Geometry check sheet. Reference: the model listing, model coordinates, mm. A direction names the side the tool comes from. Give positions to 0.01 mm unless a question says otherwise; leave off trailing zeros. Loops run counter-clockwise (first coordinate to the right, second up) from the corner with the lowest first, then second, coordinate; pieces in that order, holes last. Notation, with made-up numbers: (-4, 28.5) - (4, 28.5) arc R29 ccw to (4, 56.5) - close; hole circle Ø8 at (-20.75, 40.5). An arc over 180 degrees is marked (long way). One line per question, with ' | ' between items. Start each with the question number.
from build123d import *

# Parameters (mm, degrees)
BOSS_EXTRUDE1_DEPTH                          = 3
SKETCH11_R                                   = 1.5
CUT_EXTRUDE1_DEPTH                           = 3
CBORE_FOR_M5_HEXAGON_HEAD_BOLTS_FULL_2_COUNT = 2
CBORE_FOR_M5_HEXAGON_HEAD_BOLTS_FULL_2_PITCH = 40


with BuildPart() as part:
    # Sketch4 → Boss-Extrude1 (new body)
    with BuildSketch(Plane.XY):
        with BuildLine():
            Line((30, 0), (30, -30))
            ThreePointArc((30, -30), (0, -42.426406871), (-30, -30))
            Line((-30, -30), (-30, 0))
            ThreePointArc((-30, 0), (0, 30), (30, 0))
        make_face()
        with BuildLine():
            Line((6.2, 0), (6.2, -15.218791378))
            ThreePointArc((6.2, -15.218791378), (0, -21.418791378), (-6.2, -15.218791378))
            Line((-6.2, -15.218791378), (-6.2, 0))
            ThreePointArc((-6.2, 0), (0, 6.2), (6.2, 0))
        make_face(mode=Mode.SUBTRACT)
    extrude(amount=BOSS_EXTRUDE1_DEPTH)

    # Sketch11 → Cut-Extrude1 (cut)
    with BuildSketch(Plane.XY.offset(3)):
        with Locations((-15.463782922, 0)):
            Circle(SKETCH11_R)
        with Locations((-7.731891461, 13.392028849)):
            Circle(SKETCH11_R)
        with Locations((7.731891461, 13.392028849)):
            Circle(SKETCH11_R)
        with Locations((15.463782922, 0)):
            Circle(SKETCH11_R)
        with Locations((7.731891461, -13.392028849)):
            Circle(SKETCH11_R)
        with Locations((-7.731891461, -13.392028849)):
            Circle(SKETCH11_R)
    extrude(amount=-CUT_EXTRUDE1_DEPTH, mode=Mode.SUBTRACT)

    # Sketch14 → CBORE for M5 Hexagon head bolts-Full thread-grade C1 (revolve, cut)
    with BuildSketch(Plane(origin=(20, -30, 3), x_dir=(0, -1, 0), z_dir=(1, 0, 0))):
        Polygon((0, 0), (0, 3), (2.75, 3), (2.75, 0.5), (5.5, 0.5), (5.5, 0.025), (5.525, 0), align=None)
    cbore_for_m5_hexagon_head_bolts_full_thr = revolve(axis=Axis((20, -30, 9.35), (0, 0, -1)), mode=Mode.SUBTRACT)

    # CBORE for M5 Hexagon head bolts-Full 2: CBORE for M5 Hexagon head bolts-Full thread-grade C1 ×2
    with Locations(*[(-i * CBORE_FOR_M5_HEXAGON_HEAD_BOLTS_FULL_2_PITCH, 0, 0) for i in range(1, CBORE_FOR_M5_HEXAGON_HEAD_BOLTS_FULL_2_COUNT)]):
        add(cbore_for_m5_hexagon_head_bolts_full_thr, mode=Mode.SUBTRACT)


solid = part.part
(1) Section check D-D, the plane x = -20. Record the boundary of the cut face in (y, z) (3 decimals).
(2) Tool access check on faces 4 (the face through (7, -6, 0)), 5 (the face through (0.136, -21.417, 1.479)), 6 (the face through (-23.72, -25.95, 2.74)). Record the directions out of +Z, -Z, +X, -X, +Y, -Y that give a thin tool (end or side, any length) a straight path to the whole face; none if there is none.
(3) Section check B-B, the plane z = 1.95. Count the separate pieces of the cut face and the enclosed holes in it, and give its area (3 significant figures).
(4) Section check A-A, the plane x = 0. Record the boundary of the cut face in (y, z), and give its area (3 significant figures).
(5) Section check C-C, the plane y = 20. Record the boundary of the cut face in (x, z), and give its area (3 significant figures).
(6) Mould release check, pull along X, two halves, no side actions. Record for faces 1 (the face through (7, -6, 3)), 2 (the face through (-0.1, 6.2, 1.5)), 3 (the face through (-0.66, 29.993, 1.479)): pulls with the +X half, pulls with the -X half, needs draft (parallel to the pull), parting line crosses it, or undercut.
(7) Material ranges on line 1 (X direction, y = -30, z = 1.2); line 2 (X direction, y = -30, z = 2.7); line 3 (X direction, y = -4.5, z = 2.25), recorded low to high.
(8) Depth check by flat-ended pin: pin 1 Ø5.5 at (x, y) = (-21.5, -31) entering from +Z. Enter the tip coordinate at first touch or a pass-through.
Numbers:
1) outline: (-37.417, 0) - (-32.75, 0) - (-32.75, 2.5) - (-35.5, 2.5) - (-35.5, 2.975) - (-35.525, 3) - (-37.417, 3) - close; (-27.25, 0) - (22.361, 0) - (22.361, 3) - (-24.475, 3) - (-24.5, 2.975) - (-24.5, 2.5) - (-27.25, 2.5) - close
2) face 4: -Z, +X, -X, +Y, -Y | face 5: +Z, -Z | face 6: +Z
3) separate pieces: 1 | enclosed holes: 9 | area: 3,330 mm^2
4) outline: (-42.43, 0) - (-21.42, 0) - (-21.42, 3) - (-42.43, 3) - close; (6.2, 0) - (30, 0) - (30, 3) - (6.2, 3) - close | area: 134 mm^2
5) outline: (-22.36, 0) - (22.36, 0) - (22.36, 3) - (-22.36, 3) - close | area: 134 mm^2
6) face 1: needs draft | face 2: undercut | face 3: parting line crosses it
7) line 1: -30 to -22.75, -17.25 to 17.25, 22.75 to 30 | line 2: -30 to -25.5, -14.5 to 14.5, 25.5 to 30 | line 3: -30 to -6.2, 6.2 to 30
8) pin 1: z = 2.5
